```python
from build123d import *

# Parameters (mm, degrees)
SKETCH_1_W                   = 200
SKETCH_1_H                   = 30
EXTRUDE_1_DEPTH              = 20
HOLE_WIZARD_M8_1_D           = 9
HOLE_WIZARD_M8_1_CBORE_D     = 15
HOLE_WIZARD_M8_1_CBORE_DEPTH = 8.6


with BuildPart() as part:
    # 草图1 → 凸台-拉伸1 (new body)
    with BuildSketch(Plane.XY):
        Rectangle(SKETCH_1_W, SKETCH_1_H)
    extrude(amount=EXTRUDE_1_DEPTH)

    # M8 六角凹头螺钉的柱形沉头孔1 (through all)
    with Locations(Plane.XY.offset(20)):
        with Locations((0, 0), (90, 0), (-90, 0)):
            CounterBoreHole(HOLE_WIZARD_M8_1_D / 2, HOLE_WIZARD_M8_1_CBORE_D / 2, HOLE_WIZARD_M8_1_CBORE_DEPTH)


solid = part.part
```
The listing builds one solid part. Answer for the finished solid, in the listing's coordinates (mm). A direction names the side the tool comes from. Round coordinates to 2 decimals unless told otherwise and drop trailing zeros. Loops run counter-clockwise (first coordinate to the right, second up) from the corner with the lowest first, then second, coordinate; pieces in that order, holes last. Notation, with made-up numbers: (29.25, 29) - (41.25, 29) arc R30 ccw to (41.25, 58) - close; hole circle Ø7 at (-13.75, 64.25). An arc over 180 degrees is marked (long way). Return JSON: item names as keys, results as strings. Group by question number.
1. Which of the six approach directions +Z, -Z, +X, -X, +Y, -Y give full straight-line access (tool end or side, diameter ignored) to faces 1 (the cylindrical face through (94.496, 0.198, 5.62)), 2 (the cylindrical face through (-97.493, 0.33, 15.76))?
2. The part is cut by section B-B on x = 90. Determine the outline of the cut face in (y, z), then the cut area to 3 significant figures.
3. The part is cut by section A-A on y = 0. Determine the outline of the cut face in (x, z).
4. Consider probe 1 along Y at (x, z) = (0, 16); probe 2 along X at (y, z) = (1.75, 15.75); probe 3 along X at (y, z) = (-5.5, 16.75). Determine where each line is inside the solid, lowest interval first.
5. The part is cut by section C-C on z = 1.75. Determine the outline of the cut face in (x, y), then the cut area to 3 significant figures.
6. Each of these flat-tipped pins is pushed along its axis until it touches: P1, Ø13.5, axis at x = 90, y = 0, coming from the +Z side; P2, Ø8, axis at x = 0, y = 0, coming from the -Z side. Where does it stop, or does it pass through?
7. The mould has two halves that part along Y. Classify faces 3 (the flat face through (-1, -15, 10)), 4 (the flat face through (-1, 10, 20)), 5 (the flat face through (0, -5, 11.4)): pulls with the +Y half, pulls with the -Y half, needs draft (parallel to the pull), parting line crosses it, or undercut.
Resolved:
{
 "1": {"face 1": "+Z, -Z", "face 2": "+Z"},
 "2": {"outline": "(-15, 0) - (-4.5, 0) - (-4.5, 11.4) - (-7.5, 11.4) - (-7.5, 20) - (-15, 20) - close; (4.5, 0) - (15, 0) - (15, 20) - (7.5, 20) - (7.5, 11.4) - (4.5, 11.4) - close", "area": "368 mm²"},
 "3": {"outline": "(-100, 0) - (-94.5, 0) - (-94.5, 11.4) - (-97.5, 11.4) - (-97.5, 20) - (-100, 20) - close; (-85.5, 0) - (-4.5, 0) - (-4.5, 11.4) - (-7.5, 11.4) - (-7.5, 20) - (-82.5, 20) - (-82.5, 11.4) - (-85.5, 11.4) - close; (4.5, 0) - (85.5, 0) - (85.5, 11.4) - (82.5, 11.4) - (82.5, 20) - (7.5, 20) - (7.5, 11.4) - (4.5, 11.4) - close; (94.5, 0) - (100, 0) - (100, 20) - (97.5, 20) - (97.5, 11.4) - (94.5, 11.4) - close"},
 "4": {"probe 1": "y = -15 to -7.5, 7.5 to 15", "probe 2": "x = -100 to -97.29, -82.71 to -7.29, 7.29 to 82.71, 97.29 to 100", "probe 3": "x = -100 to -95.1, -84.9 to -5.1, 5.1 to 84.9, 95.1 to 100"},
 "5": {"outline": "(-100, -15) - (100, -15) - (100, 15) - (-100, 15) - close; hole circle Ø9 at (-90, 0); hole circle Ø9 at (0, 0); hole circle Ø9 at (90, 0)", "area": "5,810 mm²"},
 "6": {"P1": "stops at z = 11.4", "P2": "passes through"},
 "7": {"face 3": "pulls with the -Y half", "face 4": "needs draft", "face 5": "undercut"}
}
